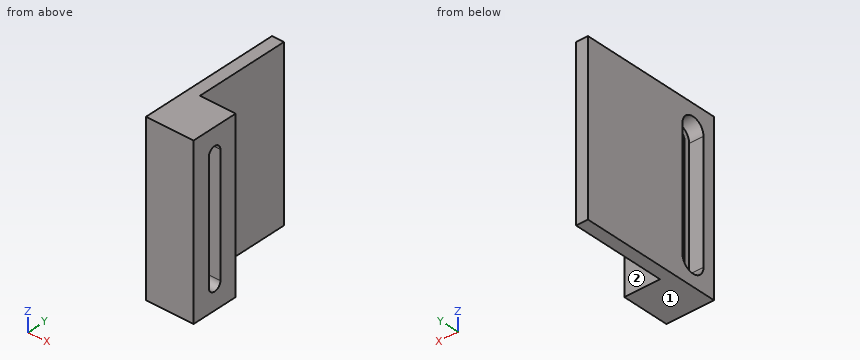
from build123d import *

# Parameters (mm, degrees)
EXTRUDE_1_DEPTH     = 70
CUT_EXTRUDE_1_DEPTH = 1200
CUT_EXTRUDE_2_DEPTH = 6


with BuildPart() as part:
    # 草图1 → 凸台-拉伸1 (new body)
    with BuildSketch(Plane.XY):
        Polygon((0, 0), (0, 60), (5, 60), (5, 20), (20, 20), (20, 0), align=None)
    extrude(amount=EXTRUDE_1_DEPTH)

    # 草图3 → 切除-拉伸1 (cut)
    with BuildSketch(Plane.ZY):
        with BuildLine():
            Line((10, 12.75), (60, 12.75))
            ThreePointArc((60, 12.75), (62.75, 10), (60, 7.25))
            Line((60, 7.25), (10, 7.25))
            ThreePointArc((10, 7.25), (7.25, 10), (10, 12.75))
        make_face()
    extrude(amount=-CUT_EXTRUDE_1_DEPTH, mode=Mode.SUBTRACT)

    # 草图6 → 切除-拉伸2 (cut)
    with BuildSketch(Plane.ZY):
        with BuildLine():
            Line((10, 5), (60, 5))
            ThreePointArc((60, 5), (65, 10), (60, 15))
            Line((60, 15), (10, 15))
            ThreePointArc((10, 15), (5, 10), (10, 5))
        make_face()
    extrude(amount=-CUT_EXTRUDE_2_DEPTH, mode=Mode.SUBTRACT)


solid = part.part
Geometry: final body of the model. Coordinates: model frame, mm. Face numbers are marked on the shaded views. A direction names the side the tool comes from. Give positions to 0.01 mm unless a question says otherwise; leave off trailing zeros. Write each loop counter-clockwise with the first axis right and the second up, starting at its lowest first coordinate (ties: lowest second). Pieces come first, ordered by that corner, then holes. Notation, with made-up numbers: (78, -3) - (112, -3) arc R28 cw to (112, 21) - close; hole circle Ø7 at (85, -38.75). An arc over 180 degrees is marked (long way). Return JSON: item names as keys, results as strings. Group by question number.
1) Line query: line 1 (Y direction, x = 16, z = 37); line 2 (Y direction, x = 1, z = 45); line 3 (Z direction, x = 7.5, y = 10). Output: solid intervals per line, ascending.
2) Set-up query: the marked faces 1 and 2. Return all of +Z, -Z, +X, -X, +Y, -Y with unobstructed straight access to the full face (end or side cutting, diameter ignored); none if empty.
3) First-contact query: P1, Ø7.5, axis at x = 10.5, z = 24.5, coming from the +Y side; P2, Ø12, axis at y = 34, z = 26, coming from the +X side; P3, Ø1.5, axis at x = 15.5, z = 47.5, coming from the -Y side. Flat tips, straight axial feed; report the tip coordinate or a pass-through.
4) Section B-B on y = 10. Return the cut outline in (x, z), plus the area to 3 significant figures.
5) Section D-D on y = 56.5. Return the cut outline in (x, z).
6) Section C-C on x = 17.75. Return the cut outline in (y, z).
7) Section A-A on z = 11. Return the cut outline in (x, y), plus the area to 3 significant figures.
Filled in:
{
 "1": {"line 1": "y = 0 to 7.25, 12.75 to 20", "line 2": "y = 0 to 5, 15 to 60", "line 3": "z = 0 to 7.25, 62.75 to 70"},
 "2": {"face 1": "-Z, +X, -X, +Y, -Y", "face 2": "+Z, -Z, +X, +Y"},
 "3": {"P1": "stops at y = 20", "P2": "stops at x = 5", "P3": "stops at y = 0"},
 "4": {"outline": "(0, 0) - (20, 0) - (20, 7.25) - (6, 7.25) - (6, 5) - (0, 5) - close; (0, 65) - (6, 65) - (6, 62.75) - (20, 62.75) - (20, 70) - (0, 70) - close", "area": "263 mm^2"},
 "5": {"outline": "(0, 0) - (5, 0) - (5, 70) - (0, 70) - close"},
 "6": {"outline": "(0, 0) - (20, 0) - (20, 70) - (0, 70) - close; hole (7.25, 10) arc R2.75 ccw to (12.75, 10) - (12.75, 60) arc R2.75 ccw to (7.25, 60) - close"},
 "7": {"outline": "(0, 0) - (20, 0) - (20, 7.25) - (6, 7.25) - (6, 5) - (0, 5) - close; (0, 15) - (6, 15) - (6, 12.75) - (20, 12.75) - (20, 20) - (5, 20) - (5, 60) - (0, 60) - close", "area": "463 mm^2"}
}
